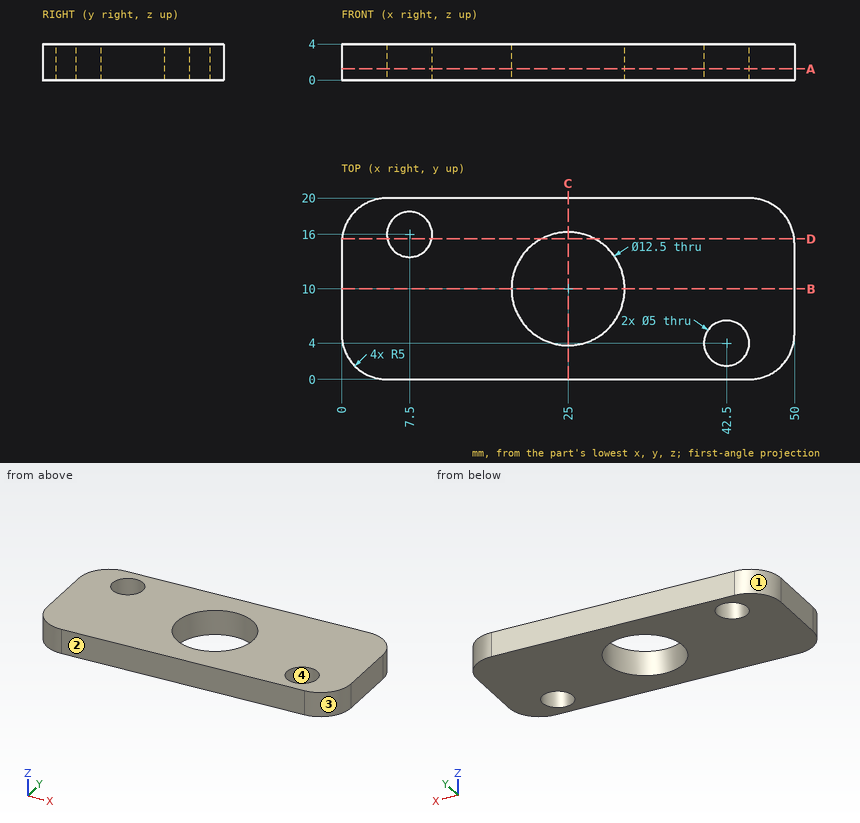
Here's the drawing with two shaded views (mm, measured from the low corner). I have some questions. Coordinates: 2 decimals unless noted, no trailing zeros. Write each loop counter-clockwise with the first axis right and the second up, starting at its lowest first coordinate (ties: lowest second). Pieces come first, ordered by that corner, then holes. Notation, with made-up numbers: (4.25, 37) - (26.25, 37) arc R24 cw to (26.25, 66) - close; hole circle Ø11 at (83.25, 39). An arc over 180 degrees is marked (long way). Return JSON: item names as keys, results as strings.
Q1. If we section it at B-B (y = 10): Please give me the cut outline in (x, z).
Computed values:
{"outline": "(0, 0) - (18.75, 0) - (18.75, 4) - (0, 4) - close; (31.25, 0) - (50, 0) - (50, 4) - (31.25, 4) - close"}
Q2. Please list where these lines run through material, in increasing order: L1, parallel to Y at x = 7.5, z = 1.1; L2, parallel to Y at x = 25, z = 2.45; L3, parallel to X at y = 15, z = 2.7. Write a range as from..to.
Computed values:
{"L1": "y = 0..13.5, 18.5..20", "L2": "y = 0..3.75, 16.25..20", "L3": "x = 0..5.21, 9.79..21.25, 28.75..50"}
Q3. Thinking about a two-plate mould opening in X: for the marked faces 1, 2, 3 and 4, which applies, +X half, -X half, draft (parallel to the pull), parting line (faces both ways), or undercut?
Computed values:
{"face 1": "-X half", "face 2": "draft", "face 3": "+X half", "face 4": "undercut"}
Q4. If we section it at D-D (y = 15.5): Please give me the cut outline in (x, z), then the cut area to 3 significant figures.
Computed values:
{"outline": "(0.03, 0) - (5.05, 0) - (5.05, 4) - (0.03, 4) - close; (9.95, 0) - (22.03, 0) - (22.03, 4) - (9.95, 4) - close; (27.97, 0) - (49.97, 0) - (49.97, 4) - (27.97, 4) - close", "area": "156 mm2"}
Q5. If we section it at C-C (x = 25): Please give me the cut outline in (y, z), then the cut area to 3 significant figures.
Computed values:
{"outline": "(0, 0) - (3.75, 0) - (3.75, 4) - (0, 4) - close; (16.25, 0) - (20, 0) - (20, 4) - (16.25, 4) - close", "area": "30.0 mm2"}
Q6. If we section it at A-A (z = 1.25): Please give me the cut outline in (x, y).
Computed values:
{"outline": "(0, 5) arc R5 ccw to (5, 0) - (45, 0) arc R5 ccw to (50, 5) - (50, 15) arc R5 ccw to (45, 20) - (5, 20) arc R5 ccw to (0, 15) - close; hole circle Ø5 at (7.5, 16); hole circle Ø12.5 at (25, 10); hole circle Ø5 at (42.5, 4)"}
